Read the model definition and answer for the solid it produces. Units are mm, in the model's axes. Coordinates: 2 decimals unless noted, no trailing zeros. Write each loop counter-clockwise with the first axis right and the second up, starting at its lowest first coordinate (ties: lowest second). Pieces come first, ordered by that corner, then holes.
1) The part is cut by section C-C (z = 1.3). Determine the outline of the cut face in (x, y).
2) The part is cut by section A-A (x = 0). Determine the outline of the cut face in (y, z).
3) Each of these flat-tipped pins is pushed along its axis until it touches: pin 1 Ø2 at (y, z) = (-7, 3.5) entering from +X; pin 2 Ø1.5 at (y, z) = (9.5, 4) entering from -X; pin 3 Ø5 at (x, y) = (-2.5, -3.5) entering from -Z; pin 4 Ø3 at (x, z) = (16.5, 3) entering from +Y. Where does it stop, or does it pass through?
4) The part is cut by section D-D (x = 6). Determine the outline of the cut face in (y, z), then the cut area to 3 significant figures.
5) The part is cut by section B-B (z = 5.1). Determine the outline of the cut face in (x, y), then the cut area to 3 significant figures.
6) Find the intervals of material crossed by line 1 (Y direction, x = 0, z = 3.2); line 2 (Y direction, x = 4, z = 3.4); line 3 (X direction, y = -4, z = 3), in increasing order.
7) Determine the mould class of faces 1 (the face through (14.93, 7.99, 0.56)), 2 (the face through (21.26, 12.23, 3.04)), 3 (the face through (0, 9.526, 3)) for opening direction X: +X half, -X half, draft (parallel to the pull), parting line (faces both ways), or undercut.
from build123d import *

# Parameters (mm, degrees)
SKETCH1_R           = 7.5
BOSS_EXTRUDE1_DEPTH = 6
SKETCH2_R           = 2.5
BOSS_EXTRUDE2_DEPTH = 15


with BuildPart() as part:
    # Sketch1 → Boss-Extrude1 (new body)
    with BuildSketch(Plane.XY):
        Polygon((-5.5, 9.526279442), (-11, 0), (-5.5, -9.526279442), (5.5, -9.526279442), (11, 0), (5.5, 9.526279442), align=None)
        Circle(SKETCH1_R, mode=Mode.SUBTRACT)
    extrude(amount=BOSS_EXTRUDE1_DEPTH)

    # Sketch2 → Boss-Extrude2 (add)
    with BuildSketch(Plane(origin=(8.25, 4.763139721, 0), x_dir=(0, 0, -1), z_dir=(0.8660254037844389, 0.49999999999999983, 0))):
        with Locations(Location((-3, 0, 0), (0, 0, 90))):
            Circle(SKETCH2_R)
    extrude(amount=BOSS_EXTRUDE2_DEPTH)


solid = part.part
Reported:
1. outline: (-11, 0) - (-5.5, -9.53) - (5.5, -9.53) - (11, 0) - (9.17, 3.18) - (22.16, 10.68) - (20.32, 13.85) - (7.33, 6.35) - (5.5, 9.53) - (-5.5, 9.53) - close; hole circle Ø15 at (0, 0)
2. outline: (-9.53, 0) - (-7.5, 0) - (-7.5, 6) - (-9.53, 6) - close; (7.5, 0) - (9.53, 0) - (9.53, 6) - (7.5, 6) - close
3. pin 1: stops at x = 7.54
3. pin 2: stops at x = -5.95
3. pin 3: passes through
3. pin 4: stops at y = 13.28
4. outline: (-8.66, 0) - (-4.5, 0) - (-4.5, 6) - (-8.66, 6) - close; (4.5, 0) - (8.66, 0) - (8.66, 6) - (4.5, 6) - close
4. area: 49.9 mm2
5. outline: (-11, 0) - (-5.5, -9.53) - (5.5, -9.53) - (11, 0) - (8.93, 3.59) - (21.92, 11.09) - (20.56, 13.44) - (7.57, 5.94) - (5.5, 9.53) - (-5.5, 9.53) - close; hole circle Ø15 at (0, 0)
5. area: 178 mm2
6. line 1: y = -9.53 to -7.5, 7.5 to 9.53
6. line 2: y = -9.53 to -6.34, 6.34 to 9.53
6. line 3: x = -8.69 to -6.34, 6.34 to 8.69
7. face 1: undercut
7. face 2: +X half
7. face 3: draft
